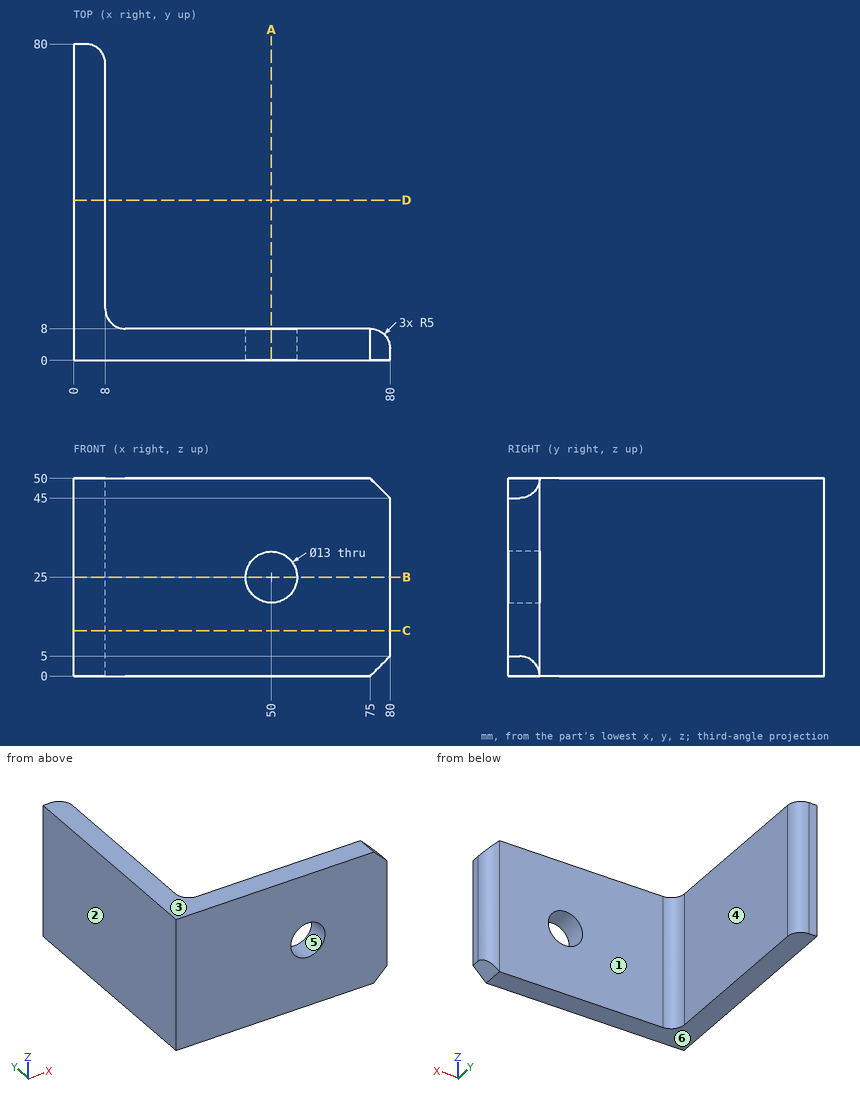
Could you check a few things on this drawing? It's one solid part, dimensions in mm from its lowest x, y, z. A direction names the side the tool comes from. Round coordinates to 2 decimals unless told otherwise and drop trailing zeros. Loops run counter-clockwise (first coordinate to the right, second up) from the corner with the lowest first, then second, coordinate; pieces in that order, holes last. Notation, with made-up numbers: M -6.5,45 L 40.5,45 A29 cw 40.5,77 Z; hole C 44.25,43.25 d6. An arc over 180 degrees is marked long. Write each question's results on one line, items separated by ' | '. Start each with the question number.
(1) I want a section at C-C (z = 11.5). Please give me the cut outline in (x, y).
(2) I want a section at B-B (z = 25). Please give me the cut outline in (x, y), then the cut area to 3 significant figures.
(3) If I drill on probe 1 along Y at (x, z) = (65.5, 14.5); probe 2 along X at (y, z) = (2.25, 25), over which ranges is the centre line in solid material (lowest first)? Write a range as from..to.
(4) Will these pins go through, and if not, where does the flat tip stop? P1, Ø6, axis at y = 68.5, z = 34.5, coming from the +X side; P2, Ø15, axis at x = 50, z = 25, coming from the -Y side; P3, Ø6, axis at x = 43.5, z = 15.5, coming from the +Y side.
(5) Thinking about a two-plate mould opening in Z: for the marked faces 3, 4, 5 and 6, which applies, pulls with the +Z half, pulls with the -Z half, needs draft (parallel to the pull), parting line crosses it, or undercut?
(6) I want a section at A-A (x = 50). Please give me the cut outline in (y, z), then the cut area to 3 significant figures.
(7) I want a section at D-D (y = 40.5). Please give me the cut outline in (x, z).
(8) On a 3-axis mill with a long thin cutter (end or side, diameter ignored), from which of +Z, -Z, +X, -X, +Y, -Y can I reach the whole of each face in a straight line? I mean the marked faces 1 and 2. Say none if no direction works.
Solved:
1) outline: M 0,0 L 80,0 L 80,3 A5 ccw 75,8 L 13,8 A5 cw 8,13 L 8,75 A5 ccw 3,80 L 0,80 Z
2) outline: M 0,0 L 43.5,0 L 43.5,8 L 13,8 A5 cw 8,13 L 8,75 A5 ccw 3,80 L 0,80 Z; M 56.5,0 L 80,0 L 80,3 A5 ccw 75,8 L 56.5,8 Z | area: 1,110 mm²
3) probe 1: y = 0..8 | probe 2: x = 0..43.5, 56.5..80
4) P1: stops at x = 8 | P2: stops at y = 0 | P3: stops at y = 8
5) face 3: pulls with the +Z half | face 4: needs draft | face 5: undercut | face 6: pulls with the -Z half
6) outline: M 0,0 L 8,0 L 8,18.5 L 0,18.5 Z; M 0,31.5 L 8,31.5 L 8,50 L 0,50 Z | area: 296 mm²
7) outline: M 0,0 L 8,0 L 8,50 L 0,50 Z
8) face 1: +Z, -Z, +X, +Y | face 2: +Z, -Z, -X, +Y, -Y
